Study the drawing (mm; zero at the part's minimum x, y, z) and answer. A direction names the side the tool comes from. Give positions to 0.01 mm unless a question says otherwise; leave off trailing zeros. Write each loop counter-clockwise with the first axis right and the second up, starting at its lowest first coordinate (ties: lowest second). Pieces come first, ordered by that corner, then holes. Notation, with made-up numbers: (79.5, -37) - (88.5, -37) arc R13 ccw to (88.5, -19) - close; hole circle Ø6 at (-10.5, -4.5). An arc over 180 degrees is marked (long way). Answer as CSV lines item,"result".
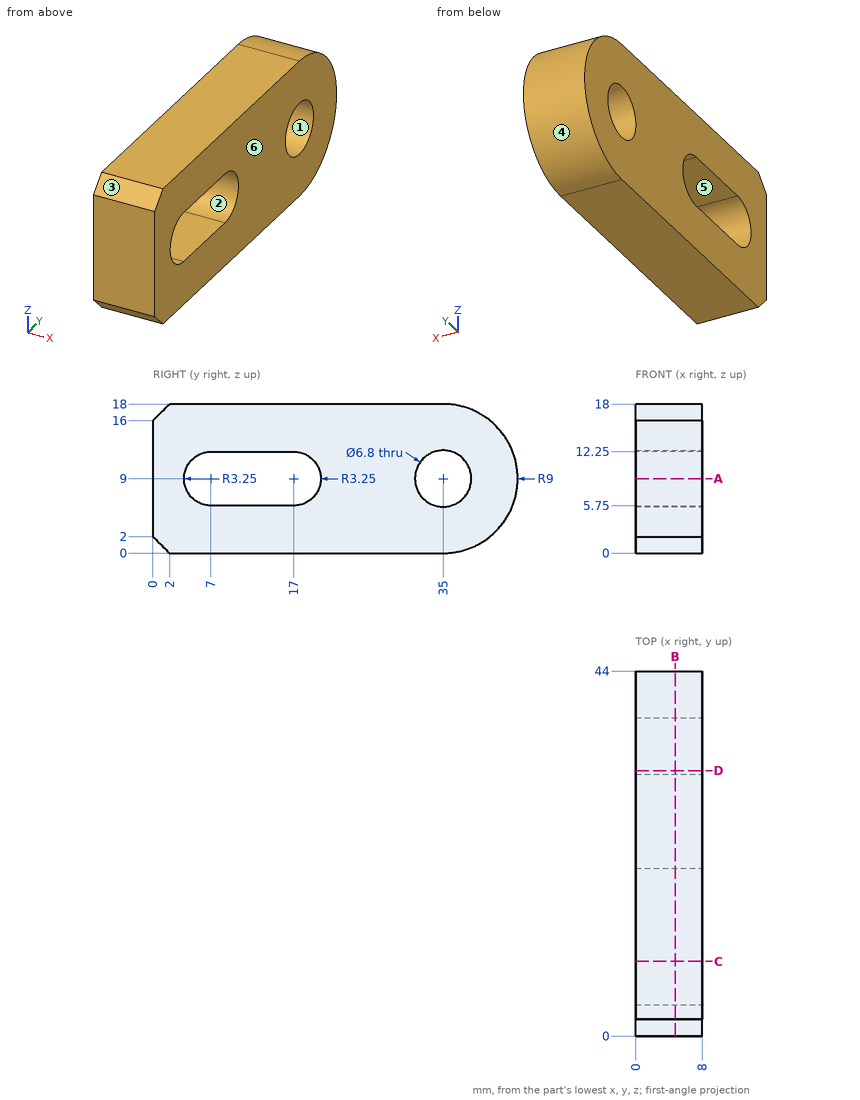
(1) This flat-tipped pin is pushed along its axis until it touches: P1, Ø3, axis at x = 5, z = 15, coming from the +Y side. Where does it stop, or does it pass through?
Worked out:
P1,"stops at y = 42.79"
(2) A cutting plane is placed at B-B (x = 4.75). Write down the section's boundary in (y, z).
Worked out:
outline,"(0, 2) - (2, 0) - (35, 0) arc R9 ccw to (35, 18) - (2, 18) - (0, 16) - close; hole (7, 5.75) - (17, 5.75) arc R3.25 ccw to (17, 12.25) - (7, 12.25) arc R3.25 ccw to start; hole circle Ø6.8 at (35, 9)"
(3) A cutting plane is placed at A-A (z = 9). Write down the section's boundary in (x, y).
Worked out:
outline,"(0, 0) - (8, 0) - (8, 3.75) - (0, 3.75) - close; (0, 20.25) - (8, 20.25) - (8, 31.6) - (0, 31.6) - close; (0, 38.4) - (8, 38.4) - (8, 44) - (0, 44) - close"
(4) The mould has two halves that part along Y. Classify the marked faces 1, 2, 3 and 4: +Y half, -Y half, draft (parallel to the pull), parting line (faces both ways), or undercut.
Worked out:
face 1,"undercut"
face 2,"undercut"
face 3,"-Y half"
face 4,"+Y half"
(5) A cutting plane is placed at C-C (y = 9). Write down the section's boundary in (x, z).
Worked out:
outline,"(0, 0) - (8, 0) - (8, 5.75) - (0, 5.75) - close; (0, 12.25) - (8, 12.25) - (8, 18) - (0, 18) - close"
(6) For the marked faces 5 and 6, determine the directions among +Z, -Z, +X, -X, +Y, -Y from which every point of the face is accessible in a straight line to the end or side of a thin tool.
Worked out:
face 5,"+X, -X"
face 6,"+Z, -Z, +X, +Y, -Y"
(7) Find the intervals of material crossed by L1, parallel to Y at x = 4.5, z = 9; L2, parallel to Z at x = 6.75, y = 7; L3, parallel to Y at x = 5.25, z = 12, in increasing order.
Worked out:
L1,"y = 0 to 3.75, 20.25 to 31.6, 38.4 to 44"
L2,"z = 0 to 5.75, 12.25 to 18"
L3,"y = 0 to 5.75, 18.25 to 33.4, 36.6 to 43.49"
(8) A cutting plane is placed at D-D (y = 32). Write down the section's boundary in (x, z), and give its area (3 significant figures).
Worked out:
outline,"(0, 0) - (8, 0) - (8, 7.4) - (0, 7.4) - close; (0, 10.6) - (8, 10.6) - (8, 18) - (0, 18) - close"
area,"118 mm^2"
